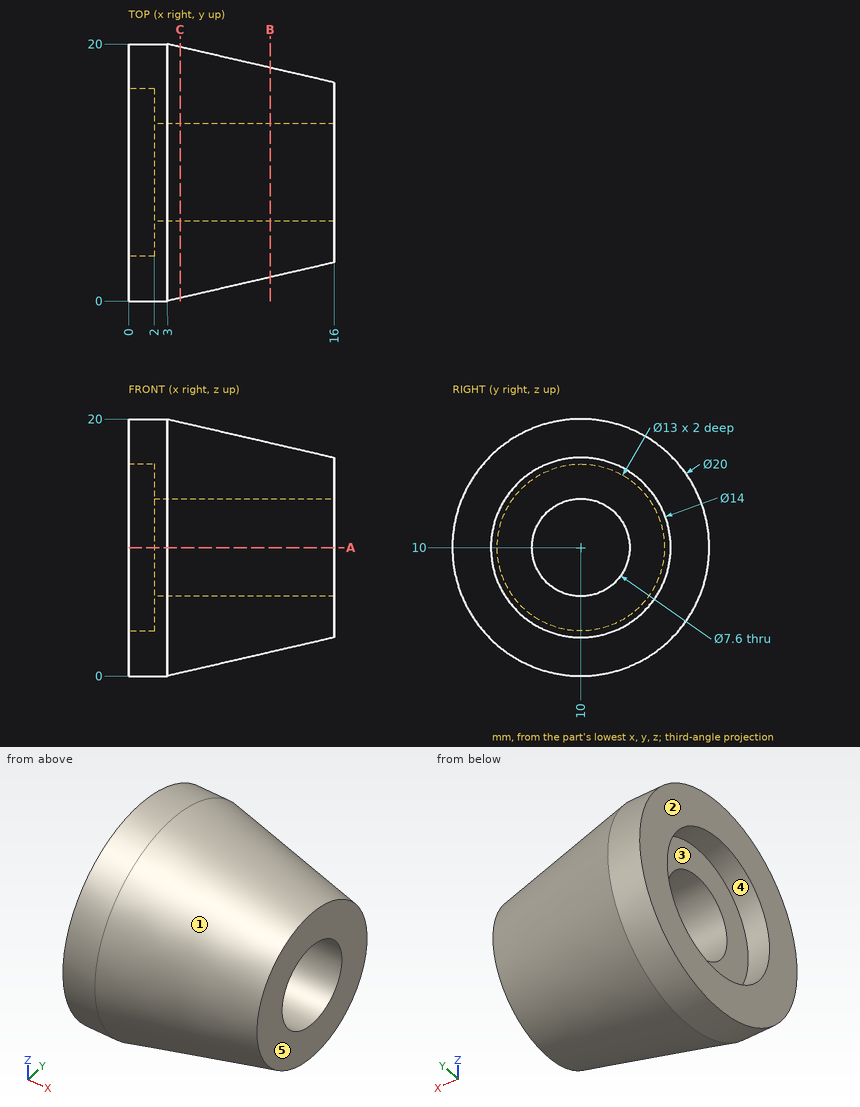
Here's the drawing with two shaded views (mm, measured from the low corner). I have some questions. A direction names the side the tool comes from. Coordinates: 2 decimals unless noted, no trailing zeros. Write each loop counter-clockwise with the first axis right and the second up, starting at its lowest first coordinate (ties: lowest second). Pieces come first, ordered by that corner, then holes. Notation, with made-up numbers: (32, 7.25) -> (45, 7.25) arc R22 cw to (45, 15.25) -> close; hole circle Ø9 at (60.25, -3). An arc over 180 degrees is marked (long way). Use a Markdown table: item, result. Add a question column.
(1) I'm going to push flat-ended pins straight in: P1, Ø12, axis at y = 10, z = 10, coming from the -X side; P2, Ø8, axis at x = 10, z = 14, coming from the +Y side; P3, Ø1.5, axis at x = 13, z = 12.5, coming from the -Y side. Where does each tip first touch, or does it pass through?
(2) If we section it at B-B, the plane x = 11: Write out the boundary of the cut face in (y, z), and give its area (3 significant figures).
(3) If we section it at C-C, the plane x = 4: Write out the boundary of the cut face in (y, z).
(4) For the marked faces 4 and 5, which set-ups out of +Z, -Z, +X, -X, +Y, -Y let a thin tool reach every point of the face, with its end or its side?
(5) We'd pull the mould along Z, two halves only. Please class the marked faces 1, 2 and 3: +Z half, -Z half, draft (parallel to the pull), parting line (faces both ways), or undercut.
(6) Please list where these lines run through material, in increasing order: line 1 (Y direction, x = 0.6, z = 10); line 2 (X direction, y = 6, z = 13.25); line 3 (Y direction, x = 13, z = 11).
(7) If we section it at A-A, the plane z = 10: Write out the boundary of the cut face in (x, y).
Outcome:
| question | item | result |
|---|---|---|
| 1 | P1 | stops at x = 2 |
| 1 | P2 | stops at y = 18.98 |
| 1 | P3 | stops at y = 2.44 |
| 2 | outline | circle Ø16.31 at (10, 10); hole circle Ø7.6 at (10, 10) |
| 2 | area | 164 mm^2 |
| 3 | outline | circle Ø19.54 at (10, 10); hole circle Ø7.6 at (10, 10) |
| 4 | face 4 | -X |
| 4 | face 5 | +Z, -Z, +X, +Y, -Y |
| 5 | face 1 | parting line |
| 5 | face 2 | draft |
| 5 | face 3 | undercut |
| 6 | line 1 | y = 0 to 3.5, 16.5 to 20 |
| 6 | line 2 | x = 2 to 16 |
| 6 | line 3 | y = 2.37 to 6.33, 13.67 to 17.63 |
| 7 | outline | (0, 0) -> (3, 0) -> (16, 3) -> (16, 6.2) -> (2, 6.2) -> (2, 3.5) -> (0, 3.5) -> close; (0, 16.5) -> (2, 16.5) -> (2, 13.8) -> (16, 13.8) -> (16, 17) -> (3, 20) -> (0, 20) -> close |
